Part model, mm, in its own coordinate system. A direction names the side the tool comes from. Coordinates: 2 decimals unless noted, no trailing zeros. Order: outer loops, then holes, each group sorted by start corner. A loop starts at its lowest first (then second) coordinate and runs counter-clockwise, first axis right, second up. Notation, with made-up numbers: M -16,17.25 L 22,17.25 A38 cw 22,56.25 Z; hole C 57,84 d10. An arc over 180 degrees is marked long. Write item = value, one per line. Start each with the question number.
from build123d import *

# Parameters (mm, degrees)
SKETCH_1_W          = 13
SKETCH_1_H          = 15
EXTRUDE_1_DEPTH     = 5
SKETCH_2_W          = 8.5
SKETCH_2_H          = 24
CUT_EXTRUDE_1_DEPTH = 10
SKETCH_3_R          = 2
CUT_EXTRUDE_2_DEPTH = 25
SKETCH_13_R         = 4
EXTRUDE_2_DEPTH     = 3
M4X0_7_1_D          = 3.3
M4X0_7_1_DEPTH      = 10.1
M4X0_7_1_TIP        = 0.991420021


with BuildPart() as part:
    # 草图1 → 凸台-拉伸1 (new, symmetric)
    with BuildSketch(Plane.XY):
        Rectangle(SKETCH_1_W, SKETCH_1_H)
    extrude(amount=EXTRUDE_1_DEPTH, both=True)

    # 草图2 → 切除-拉伸1 (cut)
    with BuildSketch(Plane.XY.offset(5)):
        with Locations((0, 7.5)):
            Rectangle(SKETCH_2_W, SKETCH_2_H)
    extrude(amount=-CUT_EXTRUDE_1_DEPTH, mode=Mode.SUBTRACT)

    # 草图3 → 切除-拉伸2 (cut)
    with BuildSketch(Plane(origin=(6.5, 0, 0), x_dir=(0, 0, -1), z_dir=(1, 0, 0))):
        with Locations((0, 3.5)):
            Circle(SKETCH_3_R)
    extrude(amount=-CUT_EXTRUDE_2_DEPTH, mode=Mode.SUBTRACT)

    # 草图13 → 凸台-拉伸2 (add)
    with BuildSketch(Plane.XZ.offset(7.5)):
        Circle(SKETCH_13_R)
    extrude(amount=EXTRUDE_2_DEPTH)

    # M4x0.7 螺纹孔1
    with Locations(Plane(origin=(0, -10.5, 0), x_dir=(-1, 0, 0), z_dir=(0, -1, 0))):
        with Locations((0, 0)):
            Hole(M4X0_7_1_D / 2, depth=M4X0_7_1_DEPTH)
            with Locations((0, 0, -(M4X0_7_1_DEPTH + M4X0_7_1_TIP / 2))):  # 118° drill point
                Cone(0, M4X0_7_1_D / 2, M4X0_7_1_TIP, mode=Mode.SUBTRACT)


solid = part.part
Item 1: Cut at C-C, the plane z = 0. Write the cut outline in (x, y).
Item 2: Flat gauge pins, fed straight in: pin 1 (5 mm diameter, centred on x = 2.5, z = -3, fed in from +Y); pin 2 (2 mm diameter, centred on x = 0.5, z = 0, fed in from -Y); pin 3 (4.5 mm diameter, centred on x = 0, z = 0, fed in from +Y). Where does each tip first touch, or does it go through?
Item 3: 3-axis set-ups, long thin cutter, end or side, ignore diameter. For faces 1 (the flat face through (-5, 7.5, 0)), 2 (the flat face through (-4.4, -7.5, 0.1)), 3 (the flat face through (-4.25, 1, 0)): which of +Z, -Z, +X, -X, +Y, -Y reach the whole face in a straight line?
Item 4: Pull direction X, two halves, no side cores. Call faces 4 (the flat face through (2, -4.5, 0)), 5 (the flat face through (6.5, 0, 0)), 6 (the flat face through (-6.5, 0, 0)), 7 (the flat face through (-2, -5, 5)): pulls with the +X half, pulls with the -X half, needs draft (parallel to the pull), parting line crosses it, or undercut.
Item 5: Cut at D-D, the plane x = 4.75. Write the cut outline in (y, z), and give its area (3 significant figures).
Item 6: Cut at A-A, the plane y = 3.5. Write the cut outline in (x, z).
Item 7: Wall check: line 1 along X through (y, z) = (-2.25, 3.75); line 2 along Y through (x, z) = (-5.85, 0); line 3 along Y through (x, z) = (-2, 4). Give the ranges that are in metal, low to high. Write a range as [from, to].
Item 8: Cut at B-B, the plane y = 6.25. Write the cut outline in (x, z).
Filled sheet:
q1.outline = M -6.5,-7.5 L -4,-7.5 L -4,-10.5 L -1.65,-10.5 L -1.65,-4.5 L -4.25,-4.5 L -4.25,1.5 L -6.5,1.5 Z; M -6.5,5.5 L -4.25,5.5 L -4.25,7.5 L -6.5,7.5 Z; M 1.65,-10.5 L 4,-10.5 L 4,-7.5 L 6.5,-7.5 L 6.5,1.5 L 4.25,1.5 L 4.25,-4.5 L 1.65,-4.5 Z; M 4.25,5.5 L 6.5,5.5 L 6.5,7.5 L 4.25,7.5 Z
q2.pin_1 = 7.5
q2.pin_2 = through
q2.pin_3 = -4.5
q3.face_1 = +Z, -Z, +X, -X, +Y
q3.face_2 = -Y
q3.face_3 = +Z, -Z, +Y
q4.face_4 = undercut
q4.face_5 = pulls with the +X half
q4.face_6 = pulls with the -X half
q4.face_7 = needs draft
q5.outline = M -7.5,-5 L 7.5,-5 L 7.5,5 L -7.5,5 Z; hole C 3.5,0 d4
q5.area = 137 mm2
q6.outline = M -6.5,-5 L -4.25,-5 L -4.25,-2 L -6.5,-2 Z; M -6.5,2 L -4.25,2 L -4.25,5 L -6.5,5 Z; M 4.25,-5 L 6.5,-5 L 6.5,-2 L 4.25,-2 Z; M 4.25,2 L 6.5,2 L 6.5,5 L 4.25,5 Z
q7.line_1 = [-6.5, -4.25], [4.25, 6.5]
q7.line_2 = [-7.5, 1.5], [5.5, 7.5]
q7.line_3 = [-7.5, -4.5]
q8.outline = M -6.5,-5 L -4.25,-5 L -4.25,5 L -6.5,5 Z; M 4.25,-5 L 6.5,-5 L 6.5,5 L 4.25,5 Z
